Input: dimensioned drawing with shaded views. Units: mm. Origin: part minimum x, y, z. Give positions to 0.01 mm unless a question says otherwise; leave off trailing zeros. Order: outer loops, then holes, each group sorted by start corner. A loop starts at its lowest first (then second) coordinate and runs counter-clockwise, first axis right, second up.
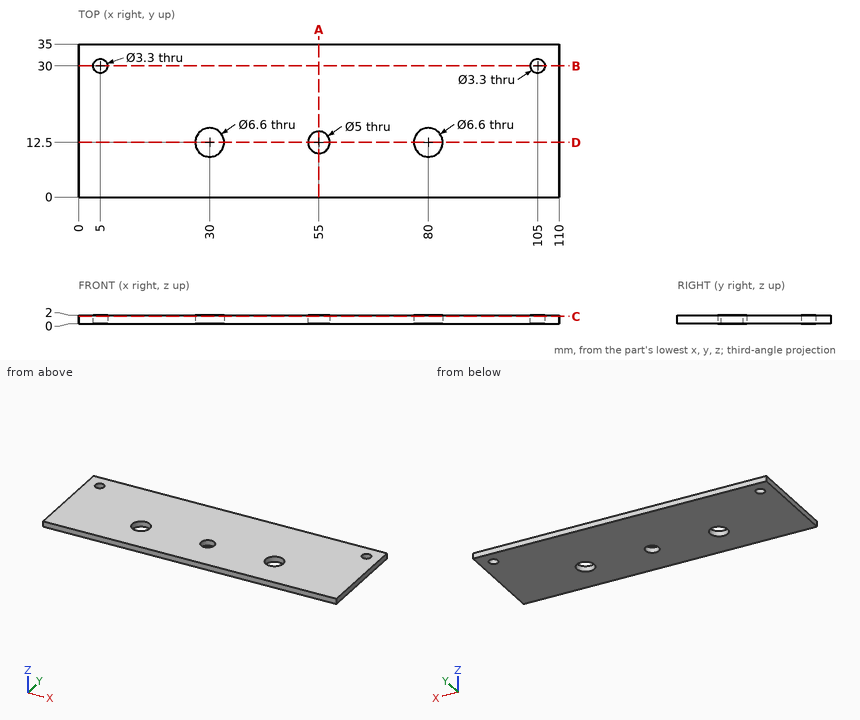
1) Section query D-D, the plane y = 12.5. Return the cut outline in (x, z).
Report:
outline: (0, 0) - (26.7, 0) - (26.7, 2) - (0, 2) - close; (33.3, 0) - (52.5, 0) - (52.5, 2) - (33.3, 2) - close; (57.5, 0) - (76.7, 0) - (76.7, 2) - (57.5, 2) - close; (83.3, 0) - (110, 0) - (110, 2) - (83.3, 2) - close
2) Section query B-B, the plane y = 30. Return the cut outline in (x, z).
Report:
outline: (0, 0) - (3.35, 0) - (3.35, 2) - (0, 2) - close; (6.65, 0) - (103.35, 0) - (103.35, 2) - (6.65, 2) - close; (106.65, 0) - (110, 0) - (110, 2) - (106.65, 2) - close
3) Material intervals for L1, parallel to Y at x = 105, z = 1.6; L2, parallel to X at y = 31, z = 0.5; L3, parallel to Y at x = 55, z = 0.5, sorted ascending.
Report:
L1: y = 0 to 28.35, 31.65 to 35
L2: x = 0 to 3.69, 6.31 to 103.69, 106.31 to 110
L3: y = 0 to 10, 15 to 35
4) Section query A-A, the plane x = 55. Return the cut outline in (y, z), and give its area (3 significant figures).
Report:
outline: (0, 0) - (10, 0) - (10, 2) - (0, 2) - close; (15, 0) - (35, 0) - (35, 2) - (15, 2) - close
area: 60.0 mm2
5) Section query C-C, the plane z = 1.7. Return the cut outline in (x, y).
Report:
outline: (0, 0) - (110, 0) - (110, 35) - (0, 35) - close; hole circle Ø3.3 at (5, 30); hole circle Ø6.6 at (30, 12.5); hole circle Ø5 at (55, 12.5); hole circle Ø6.6 at (80, 12.5); hole circle Ø3.3 at (105, 30)
